Could you check a few things on this model? Use its own coordinates, in mm. Face numbers are marked on the shaded views. Round coordinates to 2 decimals unless told otherwise and drop trailing zeros. Write each loop counter-clockwise with the first axis right and the second up, starting at its lowest first coordinate (ties: lowest second). Pieces come first, ordered by that corner, then holes. Notation, with made-up numbers: (-32, -16.75) -> (-18, -16.75) arc R17 ccw to (-18, -5.75) -> close; hole circle Ø11 at (-30.5, 29.25). An arc over 180 degrees is marked (long way). Answer in a Markdown table with one row per item.
from build123d import *

# Parameters (mm, degrees)
SKETCH_1_R          = 6.5
EXTRUDE_1_DEPTH     = 12
SKETCH_2_R          = 3
EXTRUDE_2_DEPTH     = 25
SKETCH_3_R          = 5
CUT_EXTRUDE_1_DEPTH = 0.5


with BuildPart() as part:
    # 草图1 → 凸台-拉伸1 (new body)
    with BuildSketch(Plane.XY):
        Circle(SKETCH_1_R)
    extrude(amount=EXTRUDE_1_DEPTH)

    # 草图2 → 凸台-拉伸2 (add)
    with BuildSketch(Plane.XY.offset(12)):
        Circle(SKETCH_2_R)
    extrude(amount=EXTRUDE_2_DEPTH)

    # 草图3 → 切除-拉伸1 (cut)
    with BuildSketch(Plane(origin=(0, 0, 0), x_dir=(-1, 0, 0), z_dir=(0, 0, -1))):
        Circle(SKETCH_3_R)
    extrude(amount=-CUT_EXTRUDE_1_DEPTH, mode=Mode.SUBTRACT)


solid = part.part
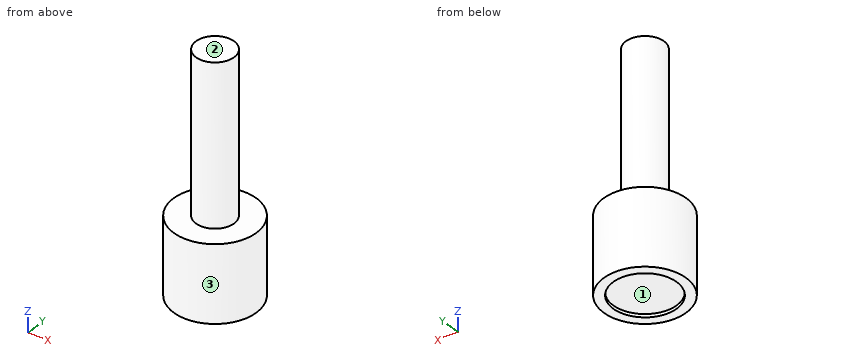
1) For pin 1 (6 mm diameter, centred on x = -5, z = 6, fed in from -Y); pin 2 (1 mm diameter, centred on x = -0.5, z = 14.5, fed in from -Y); pin 3 (2 mm diameter, centred on x = -3.5, z = 12.5, fed in from +Y); pin 4 (2 mm diameter, centred on y = -4.5, z = 25.5, fed in from -X), each with a flat end and sliding along its axis, tell me the tip position at first contact or that it passes through.
Findings:
| item | result |
|---|---|
| pin 1 | stops at y = -6.18 |
| pin 2 | stops at y = -3 |
| pin 3 | stops at y = 5.94 |
| pin 4 | passes through |
2) Imagine slicing it at A-A, the plane y = 0. Please give me the cut outline in (x, z).
Findings:
| item | result |
|---|---|
| outline | (-6.5, 0) -> (-5, 0) -> (-5, 0.5) -> (5, 0.5) -> (5, 0) -> (6.5, 0) -> (6.5, 12) -> (3, 12) -> (3, 37) -> (-3, 37) -> (-3, 12) -> (-6.5, 12) -> close |
3) Imagine slicing it at C-C, the plane z = 31. Please give me the cut outline in (x, y), plus the area to 3 significant figures.
Findings:
| item | result |
|---|---|
| outline | circle Ø6 at (0, 0) |
| area | 28.3 mm^2 |
4) Imagine slicing it at D-D, the plane x = 4. Please give me the cut outline in (y, z), plus the area to 3 significant figures.
Findings:
| item | result |
|---|---|
| outline | (-5.12, 0) -> (-3, 0) -> (-3, 0.5) -> (3, 0.5) -> (3, 0) -> (5.12, 0) -> (5.12, 12) -> (-5.12, 12) -> close |
| area | 120 mm^2 |
5) Thinking about a two-plate mould opening in X: for the marked faces 1, 2 and 3, which applies, +X half, -X half, draft (parallel to the pull), parting line (faces both ways), or undercut?
Findings:
| item | result |
|---|---|
| face 1 | undercut |
| face 2 | draft |
| face 3 | parting line |
6) Please list where these lines run through material, in increasing order: line 1 (Y direction, x = 0, z = 0.2); line 2 (Z direction, x = 5.25, y = 1.25); line 3 (Z direction, x = -1, y = 0.75).
Findings:
| item | result |
|---|---|
| line 1 | y = -6.5 to -5, 5 to 6.5 |
| line 2 | z = 0 to 12 |
| line 3 | z = 0.5 to 37 |
